Can you work these out from the model? Positions are in its coordinate system, mm. A direction names the side the tool comes from. Round coordinates to 2 decimals unless told otherwise and drop trailing zeros. Write each loop counter-clockwise with the first axis right and the second up, starting at its lowest first coordinate (ties: lowest second). Pieces come first, ordered by that corner, then holes. Notation, with made-up numbers: M 34,-37 L 40,-37 A21 ccw 40,-14 Z; hole C 45,48 d11. An arc over 180 degrees is marked long. Answer as a JSON object with one key per item and string values. Group by question number.
1) Suppose I cut it at C-C, the plane y = 6. Write out the boundary of the cut face in (x, z).
2) If we mould it in two halves opening along X, with no side actions, what happens to faces 5 (the cylindrical face through (19.066, 68.693, -34.51)), 6 (the flat face through (37.928, 53, -35)), 7 (the flat face through (89, 22, 0))? For each: +X half, -X half, draft (parallel to the pull), parting line (faces both ways), or undercut.
3) Suppose I cut it at B-B, the plane z = -49. Write out the boundary of the cut face in (x, y).
4) Suppose I cut it at D-D, the plane z = -33. State how many separate pieces and enclosed holes the cut face has, and give its area (3 significant figures).
5) I'm going to push flat-ended pins straight in: pin 1 Ø24 at (x, z) = (15, -35) entering from -Y; pin 2 Ø22.5 at (y, z) = (44.5, -50.5) entering from +X; pin 3 Ø12 at (x, z) = (119.5, -7) entering from +Y; pin 4 Ø1.5 at (x, z) = (28.5, -52) entering from -Y. Where does each tip first touch, or does it pass through?
6) On a 3-axis mill with a long thin cutter (end or side, diameter ignored), from which of +Z, -Z, +X, -X, +Y, -Y can I reach the whole of each face in a straight line? I mean faces 1 (the flat face through (89, 22, -70)), 2 (the flat face through (5, 50, -35)), 3 (the flat face through (96, 31, -12)), 4 (the flat face through (89, 19, -22)). Say none if no direction works.
7) Please list where these lines run through material, in increasing order: L1, parallel to Z at x = 150, y = 24; L2, parallel to Z at x = 44, y = 6.5; L3, parallel to X at y = 27.5, z = -10. Write a range as [from, to].
8) Suppose I cut it at A-A, the plane x = 63. Write out the boundary of the cut face in (y, z).
from build123d import *

# Parameters (mm, degrees)
BASE_BODY_DEPTH    = 70
PIN_BOSS_SKETCH_R  = 8
PIN_BOSS_DEPTH     = 28
PIN_HOLE_SKETCH_R  = 4.5
PIN_HOLE_DEPTH     = 28
END_SLOT_CUT_DEPTH = 208.754707688


with BuildPart() as part:
    # Base Profile Sketch → Base Body (new body)
    with BuildSketch(Plane.XY):
        with BuildLine():
            Line((0, 0), (180, 0))
            Line((180, 0), (180.209078325, 55.999609697))
            Line((180.209078325, 55.999609697), (152.209078325, 55.999609697))
            Line((152.209078325, 55.999609697), (152.209078325, 30.999609697))
            Line((152.209078325, 30.999609697), (37.928452135, 30.999609697))
            Line((37.928452135, 30.999609697), (37.928452135, 75.999609697))
            ThreePointArc((37.928452135, 75.999609697), (18.849811309, 68.493644543), (10, 50))
            Line((10, 50), (0, 50))
            Line((0, 50), (0, 0))
        make_face()
    extrude(amount=-BASE_BODY_DEPTH)

    # Pin Boss Sketch → Pin Boss (add)
    with BuildSketch(Plane(origin=(179.99749092, -0.67203279, 0), x_dir=(0, 0, -1), z_dir=(0.9999930303095579, -0.0037335415234940133, 0))):
        with Locations(Location((35, 56.672037474, 0), (0, 0, 90))):
            Circle(PIN_BOSS_SKETCH_R)
    extrude(amount=-PIN_BOSS_DEPTH)

    # Pin Hole Sketch → Pin Hole (cut)
    with BuildSketch(Plane(origin=(179.99749092, -0.67203279, 0), x_dir=(0, 0, -1), z_dir=(0.9999930303095579, -0.0037335415234940133, 0))):
        with Locations(Location((35, 56.672037474, 0), (0, 0, 90))):
            Circle(PIN_HOLE_SKETCH_R)
    extrude(amount=-PIN_HOLE_DEPTH, mode=Mode.SUBTRACT)

    # End Slot Sketch → End Slot Cut (cut, through all)
    with BuildSketch(Plane.ZY):
        Polygon((-52.359197148, 0), (-52.359197148, 19), (-46, 19), (-46, 41), (-24, 41), (-24, 19), (-19, 19), (-19, 0), align=None)
    extrude(amount=-END_SLOT_CUT_DEPTH, mode=Mode.SUBTRACT)


solid = part.part
Results:
{
 "1": {"outline": "M 0,-70 L 180.02,-70 L 180.02,-52.36 L 0,-52.36 Z; M 0,-19 L 180.02,-19 L 180.02,0 L 0,0 Z"},
 "2": {"face 5": "-X half", "face 6": "undercut", "face 7": "draft"},
 "3": {"outline": "M 0,19 L 180.07,19 L 180.21,56 L 152.21,56 L 152.21,31 L 37.93,31 L 37.93,76 A28 ccw 10,50 L 0,50 Z"},
 "4": {"separate pieces": "3", "enclosed holes": "0", "area": "1,310 mm^2"},
 "5": {"pin 1": "y = 19", "pin 2": "x = 180.21", "pin 3": "y = 31", "pin 4": "y = 0"},
 "6": {"face 1": "-Z, +X, -X, +Y, -Y", "face 2": "+Z, -Z, -X, +Y", "face 3": "+Z, -Z, +Y", "face 4": "+X, -X, -Y"},
 "7": {"L1": "[-70, -46], [-24, 0]", "L2": "[-70, -52.36], [-19, 0]", "L3": "[0, 180.1]"},
 "8": {"outline": "M 0,-70 L 31,-70 L 31,-46 L 19,-46 L 19,-52.36 L 0,-52.36 Z; M 0,-19 L 19,-19 L 19,-24 L 31,-24 L 31,0 L 0,0 Z"}
}
